from build123d import *


with BuildPart() as part:
    # Sketch1 → Revolve1 (revolve)
    with BuildSketch(Plane.XY, mode=Mode.PRIVATE) as revolve1_sk:
        with BuildLine():
            Line((0, 0), (0, 5))
            Line((0, 5), (-2, 7))
            Line((-2, 7), (-50, 7))
            Line((-50, 7), (-50, 10))
            Line((-50, 10), (-55, 10))
            Line((-55, 10), (-55, 7))
            Line((-55, 7), (-58, 7))
            ThreePointArc((-58, 7), (-62.949747468, 4.949747468), (-65, 0))
            Line((-65, 0), (0, 0))
        make_face()
    revolve(revolve1_sk.sketch.rotate(Axis((-89.758555814, 0, 0), (1, 0, 0)), 90), axis=Axis((-89.758555814, 0, 0), (1, 0, 0)))


solid = part.part
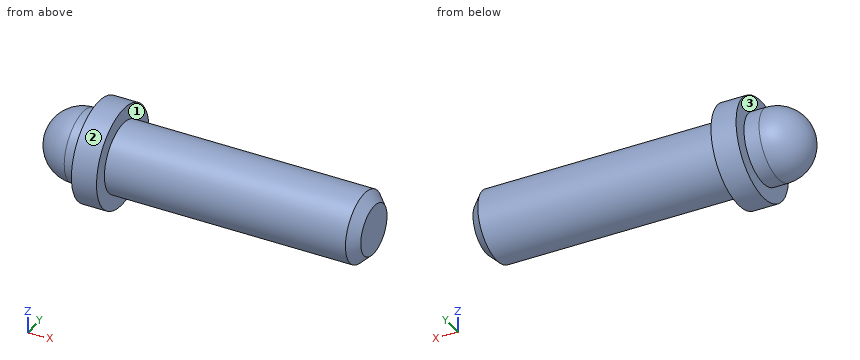
The listing builds one solid part. Answer for the finished solid, in the listing's coordinates (mm). Face numbers are marked on the shaded views. A direction names the side the tool comes from. Coordinates: 2 decimals unless noted, no trailing zeros. Write each loop counter-clockwise with the first axis right and the second up, starting at its lowest first coordinate (ties: lowest second). Pieces come first, ordered by that corner, then holes. Notation, with made-up numbers: (64.5, -4) - (79.5, -4) arc R22 ccw to (79.5, 28) - close; hole circle Ø3 at (74, 88.25). An arc over 180 degrees is marked (long way). Put each result on its own line as item: value.
1. Flat-ended cylindrical pins translate along their axes: pin 1 Ø10 at (x, z) = (-21.5, -6) entering from +Y; pin 2 Ø2 at (x, z) = (-15.5, 2.5) entering from -Y; pin 3 Ø1 at (y, z) = (-1, -3) entering from -X. Find the tip coordinate at first contact, or state that the pin passes through.
Answer sheet:
pin 1: stops at y = 6.93
pin 2: stops at y = -6.84
pin 3: stops at x = -64.47
2. The part is cut by section C-C on x = -48. Give the vertices of the cut face in (y, z).
Answer sheet:
outline: circle Ø14 at (0, 0)
3. The part is cut by section D-D on y = -7.75. Give the vertices of the cut face in (x, z).
Answer sheet:
outline: (-55, -6.32) - (-50, -6.32) - (-50, 6.32) - (-55, 6.32) - close
4. A tool of negligible diameter and unlimited length cuts with its end or side. For the marked faces 1, 2 and 3, from which of +Z, -Z, +X, -X, +Y, -Y can it reach the whole face along a straight path? Write none if from no direction.
Answer sheet:
face 1: +X
face 2: +X, -X
face 3: -X
5. Find the intervals of material crossed by line 1 along X through (y, z) = (8.5, -1); line 2 along Y through (x, z) = (-36, -5); line 3 along Z through (x, y) = (-29, 1.5), in increasing order. Write a range as from..to.
Answer sheet:
line 1: x = -55..-50
line 2: y = -4.9..4.9
line 3: z = -6.84..6.84
6. The part is cut by section A-A on y = 0. Give the vertices of the cut face in (x, z).
Answer sheet:
outline: (-58, -7) - (-55, -7) - (-55, -10) - (-50, -10) - (-50, -7) - (-2, -7) - (0, -5) - (0, 5) - (-2, 7) - (-50, 7) - (-50, 10) - (-55, 10) - (-55, 7) - (-58, 7) arc R7 ccw to start
